The model under review builds one solid part; all positions refer to its coordinate system, in mm. Face numbers are marked on the shaded views. A direction names the side the tool comes from. Round coordinates to 2 decimals unless told otherwise and drop trailing zeros. Order: outer loops, then holes, each group sorted by start corner. A loop starts at its lowest first (then second) coordinate and runs counter-clockwise, first axis right, second up. Notation, with made-up numbers: M 23,16 L 49,16 A19 cw 49,36 Z; hole C 57.5,-29.75 d1. An arc over 180 degrees is marked long. Answer as a JSON object with one key per item and string values. Group by question number.
1) Consider section B-B, the plane z = -6. Write out the cut boundary in (x, y), then the cut area to 3 significant figures.
2) For the marked faces 1, 2 and 3, list the 3-axis set-ups (+Z, -Z, +X, -X, +Y, -Y) from which the entire face can be reached by the end or side of a thin tool; tool diameter is ignored.
3) Consider section D-D, the plane x = 11.5. Write out the cut boundary in (y, z), then the cut area to 3 significant figures.
4) Consider section A-A, the plane x = 64.5. Write out the cut boundary in (y, z).
5) To check wall thickness, follow line 1 (Y direction, x = 39.75, z = 0); line 2 (Z direction, x = 6, y = -9); line 3 (Y direction, x = 40, z = 15). State the ranges of each line that lie inside material, in increasing order.
6) Consider section C-C, the plane y = 79. Write out the cut boundary in (x, z), then the cut area to 3 significant figures.
7) Insertion check: pin 1 Ø10 at (x, z) = (8, 10.5) entering from +Y; pin 2 Ø3 at (x, z) = (21, -10.5) entering from -Y; pin 3 Ø3 at (y, z) = (4, -15) entering from -X; pin 4 Ø4.5 at (y, z) = (4, 15) entering from +X. Each pin has a flat end and moves straight along its axis. Give the tip position at first contact, or say it passes through.
8) The part is to be moulded in two halves that separate along Y. For the marked faces 4, 5 and 6, say which applies: +Y half, -Y half, draft (parallel to the pull), parting line (faces both ways), or undercut.
```python
from build123d import *

# Parameters (mm, degrees)
BOSS_EXTRUDE1_DEPTH   = 20
BOSS_EXTRUDE2_DEPTH   = 4
SKETCH3_R             = 2.25
CUT_EXTRUDE2_DEPTH    = 164.343962239
M4_TAPPED_HOLE1_D     = 3.3
M4_TAPPED_HOLE2_D     = 3.3
M4_TAPPED_HOLE2_DEPTH = 11.5
M4_TAPPED_HOLE2_TIP   = 0.991420021
CUT_EXTRUDE3_REACH    = 151.937
SKETCH12_W            = 6
SKETCH12_H            = 54
M4_TAPPED_HOLE3_D     = 3.3
M4_TAPPED_HOLE3_DEPTH = 11.5
M4_TAPPED_HOLE3_TIP   = 0.991420021
CHAMFER1_SIZE         = 1
FILLET1_R             = 1
FILLET2_R             = 5


with BuildPart() as part:
    # Sketch1 → Boss-Extrude1 (new, symmetric)
    with BuildSketch(Plane.XY):
        Polygon((0, 0), (32.5, 0), (32.5, 125), (47.5, 125), (47.5, -20), (72.5, -20), (72.5, -35), (32.5, -35), (32.5, -15), (0, -15), align=None)
    extrude(amount=BOSS_EXTRUDE1_DEPTH, both=True)

    # Sketch2 → Boss-Extrude2 (add, symmetric)
    with BuildSketch(Plane.XY):
        Polygon((47.5, 125), (52.5, 125), (72.5, -5), (72.5, -20), (47.5, -20), align=None)
    extrude(amount=BOSS_EXTRUDE2_DEPTH, both=True)

    # Sketch3 → Cut-Extrude2 (cut, through all)
    with BuildSketch(Plane(origin=(0, -20, 0), x_dir=(1, 0, 0), z_dir=(0, 1, 0))):
        with Locations(Location((64.5, -12.5, 0), (0, 0, 270))):
            Circle(SKETCH3_R)
        with Locations(Location((64.5, 12.5, 0), (0, 0, 270))):
            Circle(SKETCH3_R)
    extrude(amount=-CUT_EXTRUDE2_DEPTH, mode=Mode.SUBTRACT)

    # M4 Tapped Hole1 (through all)
    with Locations(Plane(origin=(0, 0, 0), x_dir=(-1, 0, 0), z_dir=(0, 1, 0))):
        with Locations((-6, -10), (-6, 10)):
            Hole(M4_TAPPED_HOLE1_D / 2)

    # M4 Tapped Hole2
    with Locations(Plane(origin=(32.5, -167.050225356, 16.087508651), x_dir=(0, 0, 1), z_dir=(-1, 0, 0))):
        with Locations((-16.087508651, 276.050225356), (-16.087508651, 251.050225356)):
            Hole(M4_TAPPED_HOLE2_D / 2, depth=M4_TAPPED_HOLE2_DEPTH)
            with Locations((0, 0, -(M4_TAPPED_HOLE2_DEPTH + M4_TAPPED_HOLE2_TIP / 2))):  # 118° drill point
                Cone(0, M4_TAPPED_HOLE2_D / 2, M4_TAPPED_HOLE2_TIP, mode=Mode.SUBTRACT)

    # Sketch12 → Cut-Extrude3 (cut, up to next)
    with BuildSketch(Plane(origin=(0, 0, -20), x_dir=(-1, 0, 0), z_dir=(0, 0, -1)), mode=Mode.PRIVATE) as cut_extrude3_sk1:
        with Locations((-35.5, 27)):
            Rectangle(SKETCH12_W, SKETCH12_H)
    cut_extrude3_tool1 = extrude(cut_extrude3_sk1.sketch, amount=-CUT_EXTRUDE3_REACH, mode=Mode.PRIVATE) & part.part
    add(cut_extrude3_tool1.solids().sort_by_distance((35.5, 27, -20))[0], mode=Mode.SUBTRACT)

    # M4 Tapped Hole3
    with Locations(Plane.ZY.offset(-38.5)):
        with Locations((-15, 4), (15, 4)):
            Hole(M4_TAPPED_HOLE3_D / 2, depth=M4_TAPPED_HOLE3_DEPTH)
            with Locations((0, 0, -(M4_TAPPED_HOLE3_DEPTH + M4_TAPPED_HOLE3_TIP / 2))):  # 118° drill point
                Cone(0, M4_TAPPED_HOLE3_D / 2, M4_TAPPED_HOLE3_TIP, mode=Mode.SUBTRACT)

    # Chamfer1
    chamfer1_edges = [part.edges().sort_by_distance(p)[0] for p in [
        (40, 125, -20),
        (72.5, -27.5, -20),
        (0, -7.5, -20),
        (72.5, -27.5, 20),
        (32.5, -35, 0),
        (40, 125, 20),
        (0, -7.5, 20),
    ]]
    chamfer(chamfer1_edges, length=CHAMFER1_SIZE)

    # Fillet1
    fillet1_edges = [part.edges().sort_by_distance(p)[0] for p in [
        (38.5, 0, 0),
    ]]
    fillet(fillet1_edges, radius=FILLET1_R)

    # Fillet2
    fillet2_edges = [part.edges().sort_by_distance(p)[0] for p in [
        (47.5, -20, 12),
        (32.5, -15, 0),
        (47.5, -20, -12),
    ]]
    fillet(fillet2_edges, radius=FILLET2_R)


solid = part.part
```
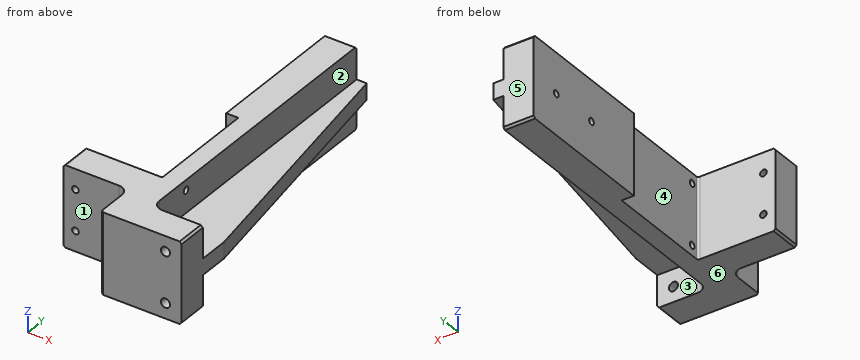
Results list:
{
 "1": {"outline": "M 0,-15 L 27.5,-15 A5 cw 32.5,-20 L 32.5,-34 L 33.5,-35 L 72.5,-35 L 72.5,-20 L 52.5,-20 A5 cw 47.5,-15 L 47.5,125 L 32.5,125 L 32.5,54 L 38.5,54 L 38.5,1 A1 cw 37.5,0 L 0,0 Z", "area": "2,950 mm^2"},
 "2": {"face 1": "+Z, -Z, -X, -Y", "face 2": "+Z, +X, +Y", "face 3": "-Z, +X, +Y"},
 "3": {"outline": "M -15,-20 L 0,-20 L 0,20 L -15,20 Z", "area": "600 mm^2"},
 "4": {"outline": "M -35,-20 L -20,-20 L -20,-14.75 L -35,-14.75 Z; M -35,-10.25 L -20,-10.25 L -20,-4 L 47,-4 L 47,4 L -20,4 L -20,10.25 L -35,10.25 Z; M -35,14.75 L -20,14.75 L -20,20 L -35,20 Z"},
 "5": {"line 1": "-35 to 82.35, 85.65 to 107.35, 110.65 to 125", "line 2": "-20 to -11.65, -8.35 to 8.35, 11.65 to 20", "line 3": "-35 to 2.35, 5.65 to 125"},
 "6": {"outline": "M 32.5,-20 L 47.5,-20 L 47.5,-4 L 59.58,-4 L 59.58,4 L 47.5,4 L 47.5,20 L 32.5,20 Z", "area": "697 mm^2"},
 "7": {"pin 1": "y = 0", "pin 2": "y = -15", "pin 3": "through", "pin 4": "x = 47.5"},
 "8": {"face 4": "undercut", "face 5": "+Y half", "face 6": "draft"}
}
